For this review, take the finished solid that the model builds, in its own axes (mm). A direction names the side the tool comes from. Give positions to 0.01 mm unless a question says otherwise; leave off trailing zeros. Loops run counter-clockwise (first coordinate to the right, second up) from the corner with the lowest first, then second, coordinate; pieces in that order, holes last. Notation, with made-up numbers: (50.25, 57) - (105.25, 57) arc R22 ccw to (105.25, 65) - close; hole circle Ø6 at (-38, 28.5). An arc over 180 degrees is marked (long way). Answer in a Markdown table with one row per item.
```python
from build123d import *

# Parameters (mm, degrees)
SKETCH1_W                      = 8
SKETCH1_H                      = 48
BOSS_EXTRUDE1_DEPTH            = 1.5
F_2_5_2_5_DIAMETER_HOLE1_D     = 2
F_2_5_2_5_DIAMETER_HOLE1_DEPTH = 5
F_2_5_2_5_DIAMETER_HOLE1_TIP   = 0.600860619
SKETCH6_W                      = 4
SKETCH6_H                      = 15
CUT_EXTRUDE1_DEPTH             = 10
SKETCH7_R                      = 1.5
CUT_EXTRUDE2_DEPTH             = 10
CHAMFER1_SIZE                  = 1
CUT_EXTRUDE3_DEPTH             = 10


with BuildPart() as part:
    # Sketch1 → Boss-Extrude1 (new body)
    with BuildSketch(Plane(origin=(0, 0, 0), x_dir=(1, 0, 0), z_dir=(0, 1, 0))):
        with Locations((4, 24)):
            Rectangle(SKETCH1_W, SKETCH1_H)
    extrude(amount=BOSS_EXTRUDE1_DEPTH)

    # Ø2.5 (2.5) Diameter Hole1
    with Locations(Plane(origin=(0, 1.5, 0), x_dir=(1, 0, 0), z_dir=(0, 1, 0))):
        with Locations((6, 46)):
            Hole(F_2_5_2_5_DIAMETER_HOLE1_D / 2, depth=F_2_5_2_5_DIAMETER_HOLE1_DEPTH)
            with Locations((0, 0, -(F_2_5_2_5_DIAMETER_HOLE1_DEPTH + F_2_5_2_5_DIAMETER_HOLE1_TIP / 2))):  # 118° drill point
                Cone(0, F_2_5_2_5_DIAMETER_HOLE1_D / 2, F_2_5_2_5_DIAMETER_HOLE1_TIP, mode=Mode.SUBTRACT)

    # Sketch6 → Cut-Extrude1 (cut)
    with BuildSketch(Plane(origin=(0, 1.5, 0), x_dir=(1, 0, 0), z_dir=(0, 1, 0))):
        with Locations((2, 40.5)):
            Rectangle(SKETCH6_W, SKETCH6_H)
    extrude(amount=-CUT_EXTRUDE1_DEPTH, mode=Mode.SUBTRACT)

    # Sketch7 → Cut-Extrude2 (cut)
    with BuildSketch(Plane(origin=(0, 1.5, 0), x_dir=(1, 0, 0), z_dir=(0, 1, 0))):
        with Locations(Location((4, 24, 0), (0, 0, 270))):
            Circle(SKETCH7_R)
        with Locations(Location((4, 8, 0), (0, 0, 270))):
            Circle(SKETCH7_R)
    extrude(amount=-CUT_EXTRUDE2_DEPTH, mode=Mode.SUBTRACT)

    # Chamfer1
    chamfer1_edges = [part.edges().sort_by_distance(p)[0] for p in [
        (0, 0.75, -33),
        (4, 0.75, -48),
        (8, 0.75, -48),
        (8, 0.75, 0),
        (0, 0.75, 0),
    ]]
    chamfer(chamfer1_edges, length=CHAMFER1_SIZE)

    # Sketch8 → Cut-Extrude3 (cut)
    with BuildSketch(Plane(origin=(0, 1.5, 0), x_dir=(1, 0, 0), z_dir=(0, 1, 0))):
        with BuildLine():
            Line((5.5, 29), (5.5, 19))
            ThreePointArc((5.5, 19), (4, 17.5), (2.5, 19))
            Line((2.5, 19), (2.5, 29))
            ThreePointArc((2.5, 29), (4, 30.5), (5.5, 29))
        make_face()
        with BuildLine():
            Line((2.5, 3), (2.5, 13))
            ThreePointArc((2.5, 13), (4, 14.5), (5.5, 13))
            Line((5.5, 13), (5.5, 3))
            ThreePointArc((5.5, 3), (4, 1.5), (2.5, 3))
        make_face()
    extrude(amount=-CUT_EXTRUDE3_DEPTH, mode=Mode.SUBTRACT)


solid = part.part
```
1. We need section C-C, the plane y = 0.85. Give the boundary of the cut face in (x, z), and give its area (3 significant figures).
Values:
| item | result |
|---|---|
| outline | (0, -32) - (1, -33) - (4, -33) - (4, -47) - (5, -48) - (7, -48) - (8, -47) - (8, -1) - (7, 0) - (1, 0) - (0, -1) - close; hole (2.5, -29) arc R1.5 ccw to (5.5, -29) - (5.5, -19) arc R1.5 ccw to (2.5, -19) - close; hole (2.5, -13) arc R1.5 ccw to (5.5, -13) - (5.5, -3) arc R1.5 ccw to (2.5, -3) - close; hole circle Ø2 at (6, -46) |
| area | 244 mm^2 |
2. Mouldability with a two-part tool opening along Z and no side actions: class faces 4 (the face through (6, 1, -48)), 5 (the face through (2.5, 1, -24)), 6 (the face through (5.5, 1, -8)), 7 (the face through (7.5, 0.7, -0.5)) as released by +Z, released by -Z, zero draft, split by the parting line, or undercut.
Values:
| item | result |
|---|---|
| face 4 | released by -Z |
| face 5 | undercut |
| face 6 | undercut |
| face 7 | released by +Z |
3. Clearance check with a flat-ended pin moving along its axis: pin 1 (1.2 mm diameter, centred on x = 6, z = -46, fed in from -Y). State where the tip first meets the part, or that it passes through.
Values:
| item | result |
|---|---|
| pin 1 | passes through |
4. Wall thickness on line 1 (X direction, y = 0.55, z = -46); line 2 (Z direction, x = 6, y = 1.15); line 3 (X direction, y = 0.25, z = -25): over which ranges is each line inside the solid? List them lowest first. Write a range as [from, to].
Values:
| item | result |
|---|---|
| line 1 | x = [4, 5], [7, 8] |
| line 2 | z = [-48, -47], [-45, 0] |
| line 3 | x = [0, 2.5], [5.5, 8] |
5. For faces 1 (the face through (2, 1, -33)), 2 (the face through (7.5, 0.7, -47.5)), 3 (the face through (4, 0.8, -14.5)), list the 3-axis set-ups (+Z, -Z, +X, -X, +Y, -Y) from which the entire face can be reached by the end or side of a thin tool; tool diameter is ignored.
Values:
| item | result |
|---|---|
| face 1 | -Z, -X, +Y, -Y |
| face 2 | -Z, +X, +Y, -Y |
| face 3 | +Y, -Y |
6. We need section A-A, the plane z = -46. Give the boundary of the cut face in (x, y), and give its area (3 significant figures).
Values:
| item | result |
|---|---|
| outline | (4, 0) - (5, 0) - (5, 1.5) - (4, 1.5) - close; (7, 0) - (8, 0) - (8, 1.5) - (7, 1.5) - close |
| area | 3.00 mm^2 |
7. We need section B-B, the plane x = 6. Give the boundary of the cut face in (y, z), and give its area (3 significant figures).
Values:
| item | result |
|---|---|
| outline | (0, -48) - (1.5, -48) - (1.5, -47) - (0, -47) - close; (0, -45) - (1.5, -45) - (1.5, 0) - (0, 0) - close |
| area | 69.0 mm^2 |
